Model file for the job. Use its own axes, mm. Face numbers are marked on the shaded views. A direction names the side the tool comes from. Coordinates: 2 decimals unless noted, no trailing zeros. Order: outer loops, then holes, each group sorted by start corner. A loop starts at its lowest first (then second) coordinate and runs counter-clockwise, first axis right, second up.
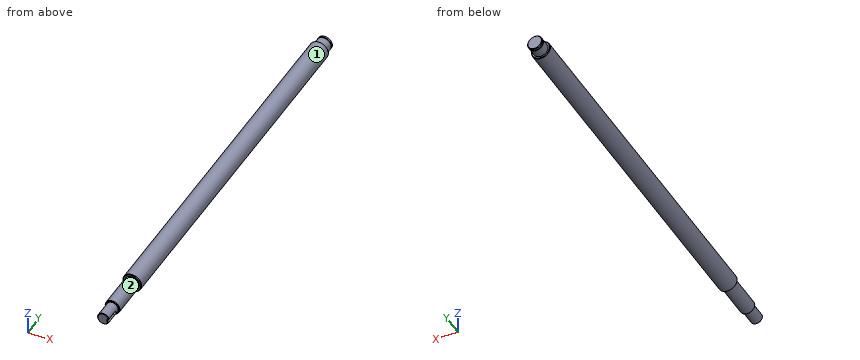
from build123d import *

# Parameters (mm, degrees)
SKETCH_5_W          = 16
SKETCH_5_H          = 619
SKETCH_6_R          = 12.5
EXTRUDE_1_DEPTH     = 65
SKETCH_7_R          = 10
EXTRUDE_2_DEPTH     = 30
EXTRUDE_START       = 20
SKETCH_8_R          = 12.5
EXTRUDE_3_DEPTH     = 20
SKETCH_9_W          = 13.903089526
SKETCH_9_H          = 1.35
CHAMFER_1_SIZE      = 1
CUT_EXTRUDE_1_DEPTH = 3.5


with BuildPart() as part:
    # 草图5 → 旋转2 (revolve)
    with BuildSketch(Plane(origin=(0, 0, 0), x_dir=(-1, 0, 0), z_dir=(0, 0, -1)), mode=Mode.PRIVATE) as revolve_2_sk:
        with Locations((-8, 15)):
            Rectangle(SKETCH_5_W, SKETCH_5_H)
    revolve(revolve_2_sk.sketch.rotate(Axis((0, -294.5, 0), (0, 1, 0)), 270), axis=Axis((0, -294.5, 0), (0, 1, 0)))

    # 草图6 → 凸台-拉伸1 (add)
    with BuildSketch(Plane.XZ.offset(294.5)):
        with Locations(Location((0, 0, 0), (0, 0, 270))):
            Circle(SKETCH_6_R)
    extrude(amount=EXTRUDE_1_DEPTH)

    # 草图7 → 凸台-拉伸2 (add)
    with BuildSketch(Plane.XZ.offset(359.5)):
        with Locations(Location((0, 0, 0), (0, 0, 270))):
            Circle(SKETCH_7_R)
    extrude(amount=EXTRUDE_2_DEPTH)

    # 草图8 → 凸台-拉伸3 (add)
    with BuildSketch(Plane(origin=(0, 324.5, 0), x_dir=(1, 0, 0), z_dir=(0, 1, 0)).offset(EXTRUDE_START)):
        with Locations(Location((0, 0, 0), (0, 0, 90))):
            Circle(SKETCH_8_R)
    extrude(amount=-EXTRUDE_3_DEPTH)

    # 草图9 → 切除-旋转1 (revolve, cut)
    with BuildSketch(Plane(origin=(0, 0, 0), x_dir=(-1, 0, 0), z_dir=(0, 0, -1)), mode=Mode.PRIVATE) as cut_revolve_1_sk:
        with Locations((18.901544763, 340.175)):
            Rectangle(SKETCH_9_W, SKETCH_9_H)
    revolve(cut_revolve_1_sk.sketch.rotate(Axis((0, 0, 0), (0, 1, 0)), 270), axis=Axis((0, 0, 0), (0, 1, 0)), mode=Mode.SUBTRACT)

    # 倒角1
    chamfer_1_edges = [part.edges().sort_by_distance(p)[0] for p in [
        (0, -359.5, 12.5),
        (0, -389.5, 10),
        (0, 344.5, 12.5),
        (0, 324.5, -16),
        (0, -294.5, -16),
    ]]
    chamfer(chamfer_1_edges, length=CHAMFER_1_SIZE)

    # 草图10 → 切除-拉伸1 (cut)
    with BuildSketch(Plane(origin=(10, 0, 0), x_dir=(0, 0, -1), z_dir=(1, 0, 0))):
        with BuildLine():
            Line((3, -369.5), (3, -402.553548126))
            ThreePointArc((3, -402.553548126), (0, -405.553548126), (-3, -402.553548126))
            Line((-3, -402.553548126), (-3, -369.5))
            ThreePointArc((-3, -369.5), (0, -366.5), (3, -369.5))
        make_face()
    extrude(amount=-CUT_EXTRUDE_1_DEPTH, mode=Mode.SUBTRACT)


solid = part.part
Q1. Which spindle directions (+Z, -Z, +X, -X, +Y, -Y) get a long thin tool onto all of the face, cutting with end or side? Do the marked faces 1 and 2. Say none if no direction does.
Established:
face 1: +Y, -Y
face 2: -Y
Q2. Probe line 1 (X direction, y = 109, z = 1); line 2 (X direction, y = 28, z = 12.5); line 3 (Y direction, x = -11, z = 0.5). List the from-to ranges inside material, lowest first.
Established:
line 1: x = -15.97 to 15.97
line 2: x = -9.99 to 9.99
line 3: y = -359.5 to 344.5
Q3. Drop flat-ended pins along their axis: P1, Ø4, axis at x = 7, z = 0, coming from the -Y side; P2, Ø3.5, axis at x = 8.5, y = -383.5, coming from the +Z side; P3, Ø4, axis at y = 183, z = -3.5, coming from the +X side; P4, Ø2.5, axis at x = 8.5, y = -384, coming from the -Z side. Give the stop position or say it passes through.
Established:
P1: stops at y = -389.5
P2: stops at z = 7.38
P3: stops at x = 15.93
P4: stops at z = -6.89
Q4. Cut at C-C, the plane y = -332. List the corners of the cut face in (x, z), plus the area to 3 significant figures.
Established:
outline: circle Ø25 at (0, 0)
area: 491 mm2
Q5. Cut at B-B, the plane y = 284.5. List the corners of the cut face in (x, z).
Established:
outline: circle Ø32 at (0, 0)
